Source: CAD feature listing. Evaluate the final solid. Frame: model axes, mm. A direction names the side the tool comes from. Coordinates: 2 decimals unless noted, no trailing zeros. Order: outer loops, then holes, each group sorted by start corner. A loop starts at its lowest first (then second) coordinate and runs counter-clockwise, first axis right, second up.
```python
from build123d import *

# Parameters (mm, degrees)
M3_TAPPED_HOLE1_D     = 2.5
M3_TAPPED_HOLE1_DEPTH = 7.5
M3_TAPPED_HOLE1_TIP   = 0.751075774
CHAMFER1_SIZE         = 0.5
M4_TAPPED_HOLE1_D     = 3.3
M4_TAPPED_HOLE1_DEPTH = 10.1
M4_TAPPED_HOLE1_TIP   = 0.991420021
M3_TAPPED_HOLE2_D     = 2.5
M3_TAPPED_HOLE2_DEPTH = 7.5
M3_TAPPED_HOLE2_TIP   = 0.751075774
M3_TAPPED_HOLE3_D     = 2.5
M3_TAPPED_HOLE3_DEPTH = 7.5
M3_TAPPED_HOLE3_TIP   = 0.751075774
M4_TAPPED_HOLE2_D     = 3.3
M4_TAPPED_HOLE2_DEPTH = 10.1
M4_TAPPED_HOLE2_TIP   = 0.991420021


with BuildPart() as part:
    # Sketch1 → Revolve1 (revolve)
    with BuildSketch(Plane.XY, mode=Mode.PRIVATE) as revolve1_sk:
        Polygon((0, 0), (40, 0), (40, 20), (32.5, 20), (32.5, 40), (0, 40), align=None)
    revolve(revolve1_sk.sketch.rotate(Axis((0, 0, 0), (0, 1, 0)), 90), axis=Axis((0, 0, 0), (0, 1, 0)))

    # Sketch2 → Cut-Revolve1 (revolve, cut)
    with BuildSketch(Plane.XY, mode=Mode.PRIVATE) as cut_revolve1_sk:
        Polygon((0, 40), (27.5, 40), (27.5, 11), (22.5, 11), (22.5, 9), (16, 9), (16, 0), (0, 0), align=None)
    revolve(cut_revolve1_sk.sketch.rotate(Axis((0, 0, 0), (0, 1, 0)), 90), axis=Axis((0, 0, 0), (0, 1, 0)), mode=Mode.SUBTRACT)

    # M3 Tapped Hole1
    with Locations(Plane(origin=(0, 40, 0), x_dir=(1, 0, 0), z_dir=(0, 1, 0))):
        with Locations((-30, 0), (-15, 25.980762114), (15, 25.980762114), (30, 0), (15, -25.980762114), (-15, -25.980762114), (0, 0)):
            Hole(M3_TAPPED_HOLE1_D / 2, depth=M3_TAPPED_HOLE1_DEPTH)
            with Locations((0, 0, -(M3_TAPPED_HOLE1_DEPTH + M3_TAPPED_HOLE1_TIP / 2))):  # 118° drill point
                Cone(0, M3_TAPPED_HOLE1_D / 2, M3_TAPPED_HOLE1_TIP, mode=Mode.SUBTRACT)

    # Chamfer1
    chamfer1_edges = [part.edges().sort_by_distance(p)[0] for p in [
        (0, 0, 40),
        (0, 20, 40),
    ]]
    chamfer(chamfer1_edges, length=CHAMFER1_SIZE)

    # M4 Tapped Hole1
    with Locations(Plane(origin=(0, 0, 0), x_dir=(-1, 0, 0), z_dir=(0, -1, 0))):
        with Locations((18.814495684, 29.412337557)):
            Hole(M4_TAPPED_HOLE1_D / 2, depth=M4_TAPPED_HOLE1_DEPTH)
            with Locations((0, 0, -(M4_TAPPED_HOLE1_DEPTH + M4_TAPPED_HOLE1_TIP / 2))):  # 118° drill point
                Cone(0, M4_TAPPED_HOLE1_D / 2, M4_TAPPED_HOLE1_TIP, mode=Mode.SUBTRACT)

    # M3 Tapped Hole2
    with Locations(Plane(origin=(0, 0, 0), x_dir=(-1, 0, 0), z_dir=(0, -1, 0))):
        with Locations((-34.334850717, 15.469705912), (-25.834850717, 0.747274048)):
            Hole(M3_TAPPED_HOLE2_D / 2, depth=M3_TAPPED_HOLE2_DEPTH)
            with Locations((0, 0, -(M3_TAPPED_HOLE2_DEPTH + M3_TAPPED_HOLE2_TIP / 2))):  # 118° drill point
                Cone(0, M3_TAPPED_HOLE2_D / 2, M3_TAPPED_HOLE2_TIP, mode=Mode.SUBTRACT)

    # M3 Tapped Hole3
    with Locations(Plane(origin=(0, 0, 0), x_dir=(-1, 0, 0), z_dir=(0, -1, 0))):
        with Locations((4.989178136, 28.35848998), (-12.331329939, 18.35848998), (-29.651838015, 8.35848998)):
            Hole(M3_TAPPED_HOLE3_D / 2, depth=M3_TAPPED_HOLE3_DEPTH)
            with Locations((0, 0, -(M3_TAPPED_HOLE3_DEPTH + M3_TAPPED_HOLE3_TIP / 2))):  # 118° drill point
                Cone(0, M3_TAPPED_HOLE3_D / 2, M3_TAPPED_HOLE3_TIP, mode=Mode.SUBTRACT)

    # M4 Tapped Hole2
    with Locations(Plane(origin=(0, 0, 0), x_dir=(-1, 0, 0), z_dir=(0, -1, 0))):
        with Locations((22.910254038, -19.681724008), (5.589745962, -29.681724008)):
            Hole(M4_TAPPED_HOLE2_D / 2, depth=M4_TAPPED_HOLE2_DEPTH)
            with Locations((0, 0, -(M4_TAPPED_HOLE2_DEPTH + M4_TAPPED_HOLE2_TIP / 2))):  # 118° drill point
                Cone(0, M4_TAPPED_HOLE2_D / 2, M4_TAPPED_HOLE2_TIP, mode=Mode.SUBTRACT)


solid = part.part
```
1. Ray query, line 1 (X direction, y = 3, z = -7.5); line 2 (Y direction, x = 36.5, z = 13.5); line 3 (Y direction, x = -16, z = 16). Return the intervals inside material, ascending.
Findings:
line 1: x = -39.29 to -14.13, 14.13 to 28.74, 30.56 to 39.29
line 2: y = 0 to 20
line 3: y = 0 to 11
2. Pin query (flat end, axial travel): P1, Ø1.5, axis at x = 30, z = 0, coming from the +Y side; P2, Ø1, axis at x = -1.5, y = 31.5, coming from the +Z side; P3, Ø5, axis at y = 11.5, z = -28.5, coming from the -X side; P4, Ø22.5, axis at x = 1, z = 1.5, coming from the +Y side. Return the tip coordinate at first contact, or that it passes through.
Findings:
P1: stops at y = 32.2
P2: stops at z = 32.48
P3: stops at x = -30.4
P4: passes through
3. Section query A-A on x = 0. Return loops of the section in (y, z).
Findings:
outline: (0, -39.5) - (0.5, -40) - (19.5, -40) - (20, -39.5) - (20, -32.5) - (40, -32.5) - (40, -27.5) - (11, -27.5) - (11, -22.5) - (9, -22.5) - (9, -16) - (0, -16) - close; (0, 16) - (9, 16) - (9, 22.5) - (11, 22.5) - (11, 27.5) - (40, 27.5) - (40, 32.5) - (20, 32.5) - (20, 39.5) - (19.5, 40) - (0.5, 40) - (0, 39.5) - close
4. Draft query along X for faces 1 (the face through (15.27, 36.2, 27.2)), 2 (the face through (5.7, 20, 32.4)), 3 (the face through (-1.76, 10.13, 39.96)). Return one class per face: released by +X, released by -X, zero draft, split by the parting line, or undercut.
Findings:
face 1: undercut
face 2: zero draft
face 3: split by the parting line
5. Section query C-C on y = 37. Return loops of the section in (x, z), plus the area to 3 significant figures.
Findings:
outline: circle Ø65 at (0, 0); hole circle Ø2.5 at (-30, 0); hole circle Ø55 at (0, 0); hole circle Ø2.5 at (-15, -25.98); hole circle Ø2.5 at (-15, 25.98); hole circle Ø2.5 at (15, -25.98); hole circle Ø2.5 at (15, 25.98); hole circle Ø2.5 at (30, 0)
area: 913 mm2
6. Access query for faces 4 (the face through (15.16, 36.2, -27.22)), 5 (the face through (15.62, 4.44, 3.47)), 6 (the face through (-24.22, 5.121, 20.686)). Directions: +Z, -Z, +X, -X, +Y, -Y. A direction counts if a zero-diameter tool reaches every point of the face in a straight line with its end or side. Return the directions, or none.
Findings:
face 4: +Y
face 5: +Y, -Y
face 6: -Y
7. Section query D-D on y = 3. Count the separate pieces of the cut face and the enclosed holes in it, plus the area to 3 significant figures.
Findings:
separate pieces: 1
enclosed holes: 9
area: 4,170 mm2
8. Section query B-B on y = 29. Return loops of the section in (x, z).
Findings:
outline: circle Ø65 at (0, 0); hole circle Ø55 at (0, 0)
